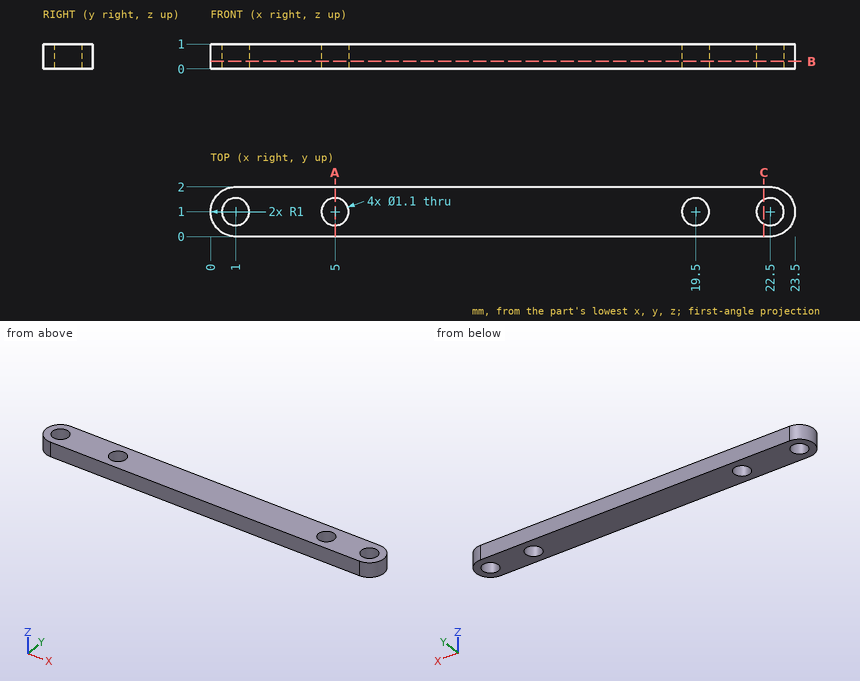
Job drawing, mm, ordinate dimensions from the low corner. One solid piece. Give positions to 0.01 mm unless a question says otherwise; leave off trailing zeros. Loops run counter-clockwise (first coordinate to the right, second up) from the corner with the lowest first, then second, coordinate; pieces in that order, holes last. Notation, with made-up numbers: (29.5, 67) -> (79.5, 67) arc R9 cw to (79.5, 73) -> close; hole circle Ø5 at (-31.5, 16). An arc over 180 degrees is marked (long way). Write each question's results on one line, items separated by ' | '.
(1) Cut at A-A on x = 5. List the corners of the cut face in (y, z).
Geometry results:
outline: (0, 0) -> (0.45, 0) -> (0.45, 1) -> (0, 1) -> close; (1.55, 0) -> (2, 0) -> (2, 1) -> (1.55, 1) -> close
(2) Cut at C-C on x = 22.25. List the corners of the cut face in (y, z).
Geometry results:
outline: (0, 0) -> (0.51, 0) -> (0.51, 1) -> (0, 1) -> close; (1.49, 0) -> (2, 0) -> (2, 1) -> (1.49, 1) -> close
(3) Cut at B-B on z = 0.3. List the corners of the cut face in (x, y).
Geometry results:
outline: (1, 0) -> (22.5, 0) arc R1 ccw to (22.5, 2) -> (1, 2) arc R1 ccw to start; hole circle Ø1.1 at (1, 1); hole circle Ø1.1 at (5, 1); hole circle Ø1.1 at (19.5, 1); hole circle Ø1.1 at (22.5, 1)
(4) Probe line 1 along Y through (x, z) = (19.5, 0.2); line 2 along X through (y, z) = (0.9, 0.65); line 3 along X through (y, z) = (1.75, 0.8). List the from-to ranges inside material, lowest first.
Geometry results:
line 1: y = 0 to 0.45, 1.55 to 2 | line 2: x = 0.01 to 0.46, 1.54 to 4.46, 5.54 to 18.96, 20.04 to 21.96, 23.04 to 23.49 | line 3: x = 0.34 to 23.16
